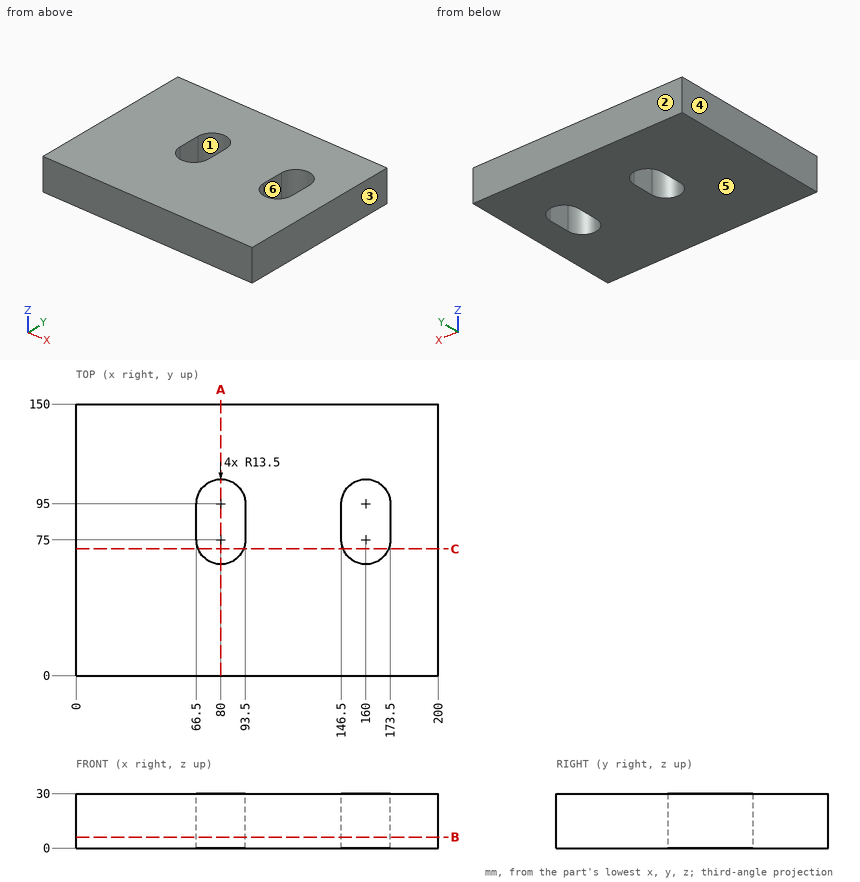
Source: three-view drawing plus pictorial views. Frame: mm from the lowest corner of the part. A direction names the side the tool comes from. Round coordinates to 2 decimals unless told otherwise and drop trailing zeros. Loops run counter-clockwise (first coordinate to the right, second up) from the corner with the lowest first, then second, coordinate; pieces in that order, holes last. Notation, with made-up numbers: (1, -16.75) -> (13, -16.75) arc R18 ccw to (13, -7.75) -> close; hole circle Ø6 at (58, -21.75). An arc over 180 degrees is marked (long way). Use one line per item in the form item = value.
Item 1: Access query for the marked faces 1 and 2. Directions: +Z, -Z, +X, -X, +Y, -Y. A direction counts if a zero-diameter tool reaches every point of the face in a straight line with its end or side. Return the directions, or none.
Evaluation:
face_1 = +Z, -Z
face_2 = +Z, -Z, +X, -X, +Y
Item 2: Material intervals for probe 1 along X at (y, z) = (85.5, 10); probe 2 along Y at (x, z) = (72, 1.5); probe 3 along X at (y, z) = (98.5, 11.75), sorted ascending.
Evaluation:
probe_1 = 0 to 66.5, 93.5 to 146.5, 173.5 to 200
probe_2 = 0 to 64.13, 105.87 to 150
probe_3 = 0 to 66.96, 93.04 to 146.96, 173.04 to 200
Item 3: Cut plane C-C on y = 70. Output: boundary loops of the cut face in (x, z), then the cut area to 3 significant figures.
Evaluation:
outline = (0, 0) -> (67.46, 0) -> (67.46, 30) -> (0, 30) -> close; (92.54, 0) -> (147.46, 0) -> (147.46, 30) -> (92.54, 30) -> close; (172.54, 0) -> (200, 0) -> (200, 30) -> (172.54, 30) -> close
area = 4,500 mm2
Item 4: Cut plane A-A on x = 80. Output: boundary loops of the cut face in (y, z).
Evaluation:
outline = (0, 0) -> (61.5, 0) -> (61.5, 30) -> (0, 30) -> close; (108.5, 0) -> (150, 0) -> (150, 30) -> (108.5, 30) -> close
Item 5: Draft query along X for the marked faces 3, 4, 5 and 6. Return one class per face: released by +X, released by -X, zero draft, split by the parting line, or undercut.
Evaluation:
face_3 = released by +X
face_4 = released by -X
face_5 = zero draft
face_6 = undercut
Item 6: Cut plane B-B on z = 6. Output: boundary loops of the cut face in (x, y).
Evaluation:
outline = (0, 0) -> (200, 0) -> (200, 150) -> (0, 150) -> close; hole (66.5, 75) arc R13.5 ccw to (93.5, 75) -> (93.5, 95) arc R13.5 ccw to (66.5, 95) -> close; hole (146.5, 75) arc R13.5 ccw to (173.5, 75) -> (173.5, 95) arc R13.5 ccw to (146.5, 95) -> close
